```python
from build123d import *

# Parameters (mm, degrees)
SKETCH_1_W          = 26.2
SKETCH_1_H          = 18.3
EXTRUDE_1_DEPTH     = 7.3
SKETCH_2_W          = 6.35
SKETCH_2_H          = 11.3
CUT_EXTRUDE_1_DEPTH = 18.567654937
SKETCH_3_W          = 4.3
SKETCH_3_H          = 7
EXTRUDE_2_DEPTH     = 9.3
SKETCH_4_W          = 13.5
SKETCH_4_H          = 3.8
CUT_EXTRUDE_2_DEPTH = 5
SKETCH_5_R          = 1.6
CUT_EXTRUDE_3_DEPTH = 19.488442336
SKETCH_6_W          = 6.920128801
SKETCH_6_H          = 1.058382597
CUT_EXTRUDE_4_DEPTH = 0.1
FILLET_1_R          = 0.5
FILLET_2_R          = 0.5


with BuildPart() as part:
    # 草图1 → 凸台-拉伸1 (new body)
    with BuildSketch(Plane.XY):
        Rectangle(SKETCH_1_W, SKETCH_1_H)
    extrude(amount=EXTRUDE_1_DEPTH)

    # 草图2 → 切除-拉伸1 (cut, through all)
    with BuildSketch(Plane.XY.offset(7.3)):
        with Locations((-9.925, -3.5)):
            Rectangle(SKETCH_2_W, SKETCH_2_H)
        with Locations((9.925, -3.5)):
            Rectangle(SKETCH_2_W, SKETCH_2_H)
    extrude(amount=-CUT_EXTRUDE_1_DEPTH, mode=Mode.SUBTRACT)

    # 草图3 → 凸台-拉伸2 (add)
    with BuildSketch(Plane.XY.offset(7.3)):
        with Locations((-4.65, 5.65)):
            Rectangle(SKETCH_3_W, SKETCH_3_H)
        with Locations((4.65, 5.65)):
            Rectangle(SKETCH_3_W, SKETCH_3_H)
    extrude(amount=EXTRUDE_2_DEPTH)

    # 草图4 → 切除-拉伸2 (cut)
    with BuildSketch(Plane.XY.offset(7.3)):
        with Locations((0, -7.25)):
            Rectangle(SKETCH_4_W, SKETCH_4_H)
    extrude(amount=-CUT_EXTRUDE_2_DEPTH, mode=Mode.SUBTRACT)

    # 草图5 → 切除-拉伸3 (cut, through all)
    with BuildSketch(Plane.XY.offset(7.3)):
        with Locations((-9.5, 5.65)):
            Circle(SKETCH_5_R)
        with Locations((9.5, 5.65)):
            Circle(SKETCH_5_R)
    extrude(amount=-CUT_EXTRUDE_3_DEPTH, mode=Mode.SUBTRACT)

    # 草图6 → 切除-拉伸4 (cut)
    with BuildSketch(Plane(origin=(-2.5, 0, 0), x_dir=(0, 0, -1), z_dir=(1, 0, 0))):
        with Locations((-10.760064401, 5.564886087)):
            Rectangle(SKETCH_6_W, SKETCH_6_H)
    cut_extrude_4 = extrude(amount=-CUT_EXTRUDE_4_DEPTH, mode=Mode.SUBTRACT)

    # 圆角1
    fillet_1_edges = [part.edges().sort_by_distance(p)[0] for p in [
        (13.1, 2.15, 3.65),
        (13.1, 9.15, 3.65),
        (-13.1, 2.15, 3.65),
        (-13.1, 9.15, 3.65),
    ]]
    fillet(fillet_1_edges, radius=FILLET_1_R)

    # 镜向1: 切除-拉伸4 across plane
    add(cut_extrude_4.mirror(Plane(origin=(0, 0, 0), x_dir=(0, 0, 1), z_dir=(1, 0, 0))), mode=Mode.SUBTRACT)

    # 圆角2
    fillet_2_edges = [part.edges().sort_by_distance(p)[0] for p in [
        (4.65, 2.15, 16.6),
        (4.65, 9.15, 16.6),
        (-4.65, 9.15, 16.6),
        (-4.65, 2.15, 16.6),
    ]]
    fillet(fillet_2_edges, radius=FILLET_2_R)


solid = part.part
```
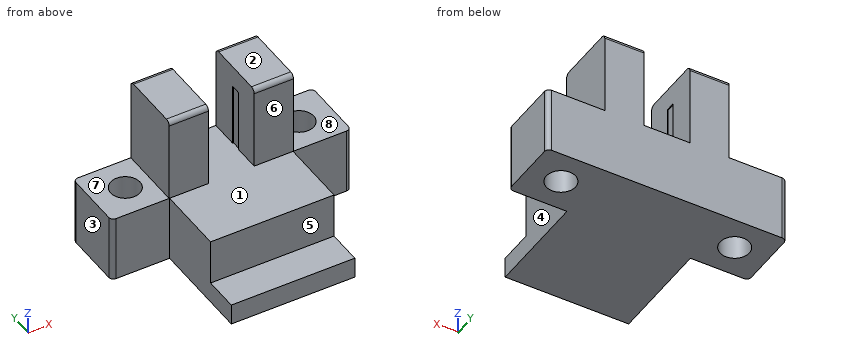
The model under review builds one solid part; all positions refer to its coordinate system, in mm. Face numbers are marked on the shaded views. A direction names the side the tool comes from. Give positions to 0.01 mm unless a question says otherwise; leave off trailing zeros. Loops run counter-clockwise (first coordinate to the right, second up) from the corner with the lowest first, then second, coordinate; pieces in that order, holes last. Notation, with made-up numbers: (-32.5, 34) - (-22.5, 34) arc R15 cw to (-22.5, 54) - close; hole circle Ø5 at (42, 8). An arc over 180 degrees is marked (long way). Answer as a JSON object with one key per item and string values.
Q1. Mouldability with a two-part tool opening along X and no side actions: class the marked faces 1, 2 and 3 as +X half, -X half, draft (parallel to the pull), parting line (faces both ways), or undercut.
Worked out:
{"face 1": "undercut", "face 2": "draft", "face 3": "-X half"}
Q2. Add section A-A on y = 5.65. State the section outline as (x, z) points.
Worked out:
{"outline": "(-13.1, 0) - (-11.1, 0) - (-11.1, 7.3) - (-13.1, 7.3) - close; (-7.9, 0) - (7.9, 0) - (7.9, 7.3) - (6.8, 7.3) - (6.8, 16.6) - (2.5, 16.6) - (2.5, 14.22) - (2.6, 14.22) - (2.6, 7.3) - (-2.6, 7.3) - (-2.6, 14.22) - (-2.5, 14.22) - (-2.5, 16.6) - (-6.8, 16.6) - (-6.8, 7.3) - (-7.9, 7.3) - close; (11.1, 0) - (13.1, 0) - (13.1, 7.3) - (11.1, 7.3) - close"}
Q3. For the marked faces 4, 5, 6, 7 and 8, list the 3-axis set-ups (+Z, -Z, +X, -X, +Y, -Y) from which the entire face can be reached by the end or side of a thin tool; tool diameter is ignored.
Worked out:
{"face 4": "+Z, -Z, +X, -Y", "face 5": "+Z, +X, -X, -Y", "face 6": "+Z, +X, -Y", "face 7": "+Z, -X, +Y, -Y", "face 8": "+Z, +X, +Y, -Y"}
Q4. Add section D-D on z = 10. State the section outline as (x, y) points.
Worked out:
{"outline": "(-6.8, 2.15) - (-2.5, 2.15) - (-2.5, 5.04) - (-2.6, 5.04) - (-2.6, 6.09) - (-2.5, 6.09) - (-2.5, 9.15) - (-6.8, 9.15) - close; (2.5, 2.15) - (6.8, 2.15) - (6.8, 9.15) - (2.5, 9.15) - (2.5, 6.09) - (2.6, 6.09) - (2.6, 5.04) - (2.5, 5.04) - close"}
Q5. Add section C-C on z = 3.5. State the section outline as (x, y) points, plus the area to 3 significant figures.
Worked out:
{"outline": "(-13.1, 2.65) arc R0.5 ccw to (-12.6, 2.15) - (-6.75, 2.15) - (-6.75, -5.35) - (6.75, -5.35) - (6.75, 2.15) - (12.6, 2.15) arc R0.5 ccw to (13.1, 2.65) - (13.1, 8.65) arc R0.5 ccw to (12.6, 9.15) - (-12.6, 9.15) arc R0.5 ccw to (-13.1, 8.65) - close; hole circle Ø3.2 at (-9.5, 5.65); hole circle Ø3.2 at (9.5, 5.65)", "area": "268 mm^2"}
Q6. Add section B-B on x = -9.5. State the section outline as (y, z) points, plus the area to 3 significant figures.
Worked out:
{"outline": "(2.15, 0) - (4.05, 0) - (4.05, 7.3) - (2.15, 7.3) - close; (7.25, 0) - (9.15, 0) - (9.15, 7.3) - (7.25, 7.3) - close", "area": "27.7 mm^2"}
Q7. To check wall thickness, follow line 1 along Y through (x, z) = (9.5, 3.25); line 2 along X through (y, z) = (4.75, 4.5); line 3 along Z through (x, y) = (-11.5, 8.25). State the ranges of each line that lie inside material, in increasing order.
Worked out:
{"line 1": "y = 2.15 to 4.05, 7.25 to 9.15", "line 2": "x = -13.1 to -10.82, -8.18 to 8.18, 10.82 to 13.1", "line 3": "z = 0 to 7.3"}
Q8. Insertion check: pin 1 (3.5 mm diameter, centred on y = 4.5, z = 11, fed in from -X); pin 2 (10 mm diameter, centred on x = 10, y = 1, fed in from +Z); pin 3 (5 mm diameter, centred on x = 8.5, y = -1, fed in from +Z); pin 4 (3.5 mm diameter, centred on y = 4, z = 12, fed in from +X). Each pin has a flat end and moves straight along its axis. Give the tip position at first contact, or say it passes through.
Worked out:
{"pin 1": "stops at x = -6.8", "pin 2": "stops at z = 16.6", "pin 3": "stops at z = 7.3", "pin 4": "stops at x = 6.8"}
